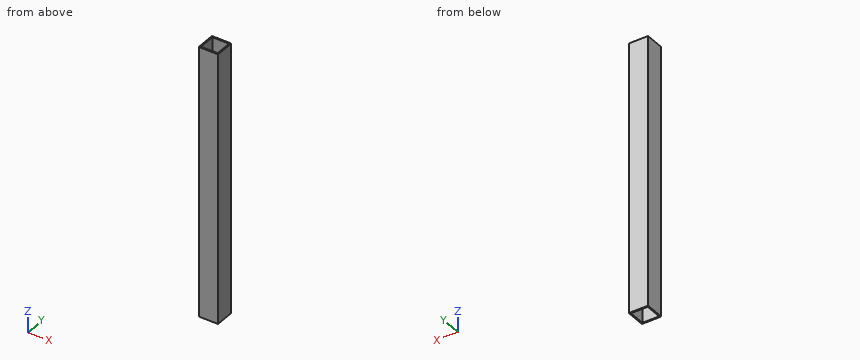
```python
from build123d import *

# Parameters (mm, degrees)
SKETCH_1_W      = 30
SKETCH_1_H      = 30
SKETCH_1_W_2    = 26
SKETCH_1_H_2    = 26
EXTRUDE_1_DEPTH = 210


with BuildPart() as part:
    # 草图1 → 凸台-拉伸1 (new, symmetric)
    with BuildSketch(Plane.XY):
        Rectangle(SKETCH_1_W, SKETCH_1_H)
        Rectangle(SKETCH_1_W_2, SKETCH_1_H_2, mode=Mode.SUBTRACT)
    extrude(amount=EXTRUDE_1_DEPTH, both=True)


solid = part.part
```
Geometry check sheet. Reference: the model listing, model coordinates, mm. Coordinates: 2 decimals unless noted, no trailing zeros. Order: outer loops, then holes, each group sorted by start corner. A loop starts at its lowest first (then second) coordinate and runs counter-clockwise, first axis right, second up.
Item 1: Section check A-A (y = 1.25). Enter the section's corners in (x, z), plus the area to 3 significant figures.
Item 2: Depth check by flat-ended pin: pin 1 (12 mm diameter, centred on x = -11, y = -3.5, fed in from +Z). Enter the tip coordinate at first touch or a pass-through.
Item 3: Section check C-C (z = 152). Enter the section's corners in (x, y), plus the area to 3 significant figures.
Item 4: Scan line: line 1 along Y through (x, z) = (-8.5, -117.5). Record every from-to range of solid material in increasing order.
Check sheet entries:
1. outline: (-15, -210) - (-13, -210) - (-13, 210) - (-15, 210) - close; (13, -210) - (15, -210) - (15, 210) - (13, 210) - close
1. area: 1,680 mm2
2. pin 1: stops at z = 210
3. outline: (-15, -15) - (15, -15) - (15, 15) - (-15, 15) - close; hole (-13, -13) - (13, -13) - (13, 13) - (-13, 13) - close
3. area: 224 mm2
4. line 1: y = -15 to -13, 13 to 15
